Source: three-view drawing plus pictorial views. Frame: mm from the lowest corner of the part. A direction names the side the tool comes from. Give positions to 0.01 mm unless a question says otherwise; leave off trailing zeros. Loops run counter-clockwise (first coordinate to the right, second up) from the corner with the lowest first, then second, coordinate; pieces in that order, holes last. Notation, with made-up numbers: M 3,25 L 42,25 A28 cw 42,44 Z; hole C 75,-40 d9. An arc over 180 degrees is marked long. Write item = value, one per line.
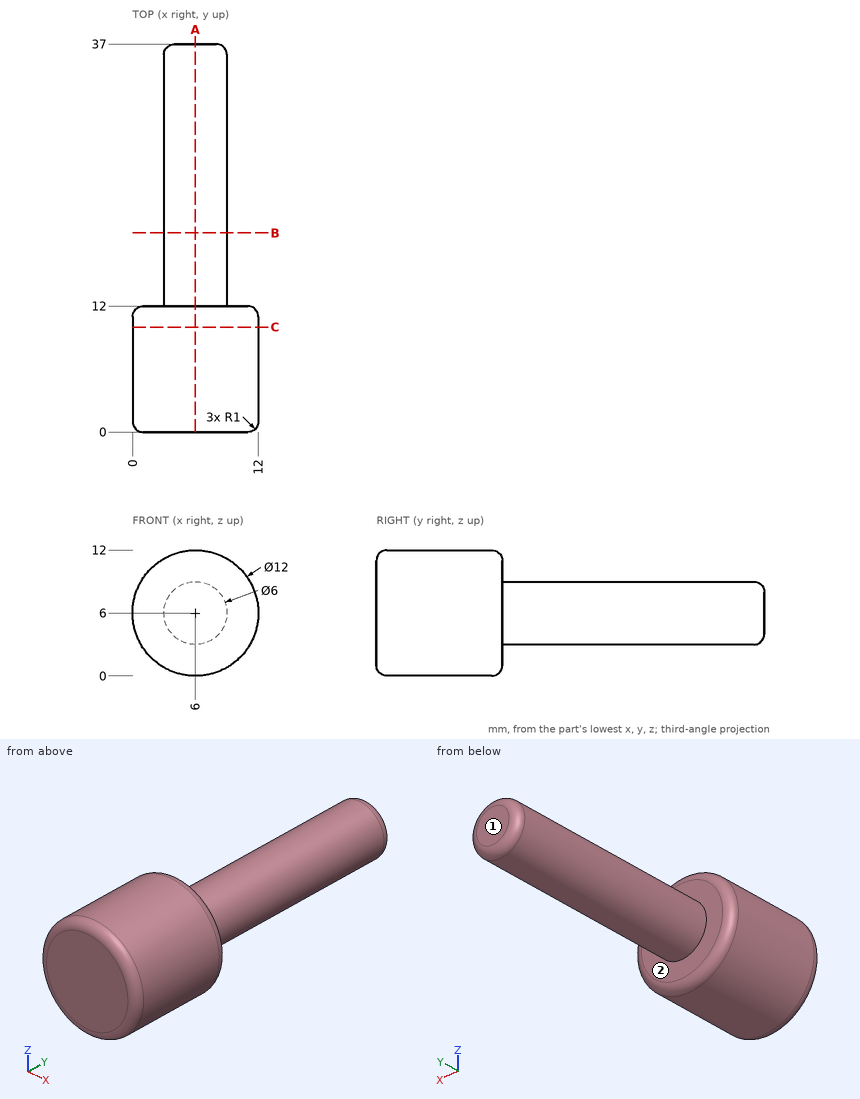
1. Cut plane B-B, the plane y = 19. Return the cut outline in (x, z), then the cut area to 3 significant figures.
Derived:
outline = C 6,6 d6
area = 28.3 mm²
2. Material intervals for probe 1 along Y at (x, z) = (7.5, 2.5); probe 2 along X at (y, z) = (11, 4); probe 3 along X at (y, z) = (29, 5), sorted ascending. Write a range as from..to.
Derived:
probe_1 = 0..12
probe_2 = 0.34..11.66
probe_3 = 3.17..8.83
3. Reachability of the marked faces 1 and 2 from +Z, -Z, +X, -X, +Y, -Y: full face, straight path, thin tool, end or side. Return the list, or none.
Derived:
face_1 = +Z, -Z, +X, -X, +Y
face_2 = +Y
4. Cut plane C-C, the plane y = 10. Return the cut outline in (x, z), then the cut area to 3 significant figures.
Derived:
outline = C 6,6 d12
area = 113 mm²
5. First-contact query: pin 1 Ø1.5 at (y, z) = (31, 7) entering from +X; pin 2 Ø6 at (y, z) = (9.5, 2) entering from +X; pin 3 Ø1.5 at (y, z) = (9, 3) entering from +X. Flat tips, straight axial feed; report the tip coordinate or a pass-through.
Derived:
pin_1 = 8.99
pin_2 = 11.92
pin_3 = 11.56
6. Cut plane A-A, the plane x = 6. Return the cut outline in (y, z), then the cut area to 3 significant figures.
Derived:
outline = M 0,1 A1 ccw 1,0 L 11,0 A1 ccw 12,1 L 12,3 L 36,3 A1 ccw 37,4 L 37,8 A1 ccw 36,9 L 12,9 L 12,11 A1 ccw 11,12 L 1,12 A1 ccw 0,11 Z
area = 293 mm²
